Source: CAD feature listing. Evaluate the final solid. Frame: model axes, mm. Round coordinates to 2 decimals unless told otherwise and drop trailing zeros. Order: outer loops, then holes, each group sorted by start corner. A loop starts at its lowest first (then second) coordinate and runs counter-clockwise, first axis right, second up. Notation, with made-up numbers: (78, -39) - (108, -39) arc R9 ccw to (108, -27) - close; hole circle Ø9 at (23, 32.25). An arc over 180 degrees is marked (long way). Return JSON: item names as keys, results as strings. Group by question number.
1) Contact query for a flat-ended pin moving along its axis: P1, Ø3, axis at x = 10, y = -45.5, coming from the -Z side. Output: stop coordinate, or through.
2) Section A-A, the plane y = 47. Return loops of the section in (x, z).
3) Section B-B, the plane x = 0. Return loops of the section in (y, z).
4) Section C-C, the plane z = 7. Return loops of the section in (x, y).
5) Mould query, pull axis X, two halves, no side actions, for faces 1 (the cylindrical face through (-5.42, 22.594, 6.084)), 2 (the flat face through (-30, -1, 6)), 3 (the flat face through (0, -80, 6)). Classes: pulls with the +X half, pulls with the -X half, needs draft (parallel to the pull), parting line crosses it, or undercut.
6) Ray query, line 1 (Y direction, x = 0, z = 8.5); line 2 (Y direction, x = 16, z = 6); line 3 (X direction, y = 37.5, z = 7.5). Return the intervals inside material, ascending. Write a range as from..to.
```python
from build123d import *

# Parameters (mm, degrees)
SKETCH_1_W          = 60
SKETCH_1_H          = 160
EXTRUDE_1_DEPTH     = 12
SKETCH_2_R          = 25
CUT_EXTRUDE_1_DEPTH = 87.27861844


with BuildPart() as part:
    # 草图1 → 凸台-拉伸1 (new body)
    with BuildSketch(Plane.XY):
        Rectangle(SKETCH_1_W, SKETCH_1_H)
    extrude(amount=EXTRUDE_1_DEPTH)

    # 草图2 → 切除-拉伸1 (cut, through all)
    with BuildSketch(Plane.XY.offset(12)):
        with Locations((0, 47)):
            Circle(SKETCH_2_R)
    extrude(amount=-CUT_EXTRUDE_1_DEPTH, mode=Mode.SUBTRACT)


solid = part.part
```
Geometry check:
{
 "1": {"P1": "z = 0"},
 "2": {"outline": "(-30, 0) - (-25, 0) - (-25, 12) - (-30, 12) - close; (25, 0) - (30, 0) - (30, 12) - (25, 12) - close"},
 "3": {"outline": "(-80, 0) - (22, 0) - (22, 12) - (-80, 12) - close; (72, 0) - (80, 0) - (80, 12) - (72, 12) - close"},
 "4": {"outline": "(-30, -80) - (30, -80) - (30, 80) - (-30, 80) - close; hole circle Ø50 at (0, 47)"},
 "5": {"face 1": "undercut", "face 2": "pulls with the -X half", "face 3": "needs draft"},
 "6": {"line 1": "-80..22, 72..80", "line 2": "-80..27.79, 66.21..80", "line 3": "-30..-23.12, 23.12..30"}
}
